The model under review builds one solid part; all positions refer to its coordinate system, in mm. Face numbers are marked on the shaded views. A direction names the side the tool comes from. Give positions to 0.01 mm unless a question says otherwise; leave off trailing zeros. Write each loop counter-clockwise with the first axis right and the second up, starting at its lowest first coordinate (ties: lowest second). Pieces come first, ordered by that corner, then holes.
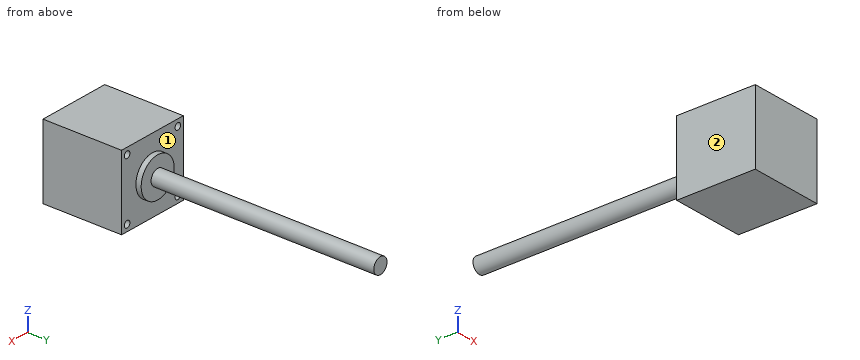
from build123d import *

# Parameters (mm, degrees)
SKETCH1_W             = 28
SKETCH1_H             = 28
BOSS_EXTRUDE1_DEPTH   = 30
SKETCH2_R             = 7.5
BOSS_EXTRUDE2_DEPTH   = 2
SKETCH3_R             = 3
BOSS_EXTRUDE3_DEPTH   = 85
SKETCH4_R             = 1
CUT_EXTRUDE1_DEPTH    = 3
M3_TAPPED_HOLE1_D     = 2.5
M3_TAPPED_HOLE1_DEPTH = 7.5
M3_TAPPED_HOLE1_TIP   = 0.751075774


with BuildPart() as part:
    # Sketch1 → Boss-Extrude1 (new body)
    with BuildSketch(Plane(origin=(0, 0, 0), x_dir=(1, 0, 0), z_dir=(0, 1, 0))):
        Rectangle(SKETCH1_W, SKETCH1_H)
    extrude(amount=BOSS_EXTRUDE1_DEPTH)

    # Sketch2 → Boss-Extrude2 (add)
    with BuildSketch(Plane(origin=(0, 30, 0), x_dir=(1, 0, 0), z_dir=(0, 1, 0))):
        with Locations(Location((0, 0, 0), (0, 0, 270))):
            Circle(SKETCH2_R)
    extrude(amount=BOSS_EXTRUDE2_DEPTH)

    # Sketch3 → Boss-Extrude3 (add)
    with BuildSketch(Plane(origin=(0, 32, 0), x_dir=(1, 0, 0), z_dir=(0, 1, 0))):
        with Locations(Location((0, 0, 0), (0, 0, 270))):
            Circle(SKETCH3_R)
    extrude(amount=BOSS_EXTRUDE3_DEPTH)

    # Sketch4 → Cut-Extrude1 (cut)
    with BuildSketch(Plane(origin=(0, 30, 0), x_dir=(1, 0, 0), z_dir=(0, 1, 0))):
        with Locations(Location((-11.5, -11.5, 0), (0, 0, 270))):
            Circle(SKETCH4_R)
        with Locations(Location((11.5, -11.5, 0), (0, 0, 270))):
            Circle(SKETCH4_R)
        with Locations(Location((-11.5, 11.5, 0), (0, 0, 270))):
            Circle(SKETCH4_R)
        with Locations(Location((11.5, 11.5, 0), (0, 0, 270))):
            Circle(SKETCH4_R)
    extrude(amount=-CUT_EXTRUDE1_DEPTH, mode=Mode.SUBTRACT)

    # M3 Tapped Hole1
    with Locations(Plane(origin=(0, 30, 0), x_dir=(1, 0, 0), z_dir=(0, 1, 0))):
        with Locations((-11.5, -11.5), (11.5, -11.5), (-11.5, 11.5), (11.5, 11.5)):
            Hole(M3_TAPPED_HOLE1_D / 2, depth=M3_TAPPED_HOLE1_DEPTH)
            with Locations((0, 0, -(M3_TAPPED_HOLE1_DEPTH + M3_TAPPED_HOLE1_TIP / 2))):  # 118° drill point
                Cone(0, M3_TAPPED_HOLE1_D / 2, M3_TAPPED_HOLE1_TIP, mode=Mode.SUBTRACT)


solid = part.part
1) Insertion check: pin 1 (1.5 mm diameter, centred on x = -11.5, z = -11.5, fed in from +Y); pin 2 (6 mm diameter, centred on y = 46, z = 1, fed in from +X); pin 3 (2 mm diameter, centred on x = 11.5, z = -11.5, fed in from +Y). Each pin has a flat end and moves straight along its axis. Give the tip position at first contact, or say it passes through.
2) Tool access review of the marked faces 1 and 2: name each direction out of +Z, -Z, +X, -X, +Y, -Y from which nothing blocks a thin tool from reaching the whole face with its end or side.
3) Consider section B-B, the plane x = -6.25. Give the boundary of the cut face in (y, z).
4) Consider section C-C, the plane y = 86. Give the boundary of the cut face in (x, z).
5) Consider section A-A, the plane z = 4.5. Give the boundary of the cut face in (x, y), then the cut area to 3 significant figures.
6) To check wall thickness, follow probe 1 along Z at (x, y) = (11.5, 26.5); probe 2 along Y at (x, z) = (-3.5, -11.5). State the ranges of each line that lie inside material, in increasing order.
7) Consider section D-D, the plane z = 0. Give the boundary of the cut face in (x, y), then the cut area to 3 significant figures.
Answer block:
1. pin 1: stops at y = 22.2
1. pin 2: stops at x = 3
1. pin 3: stops at y = 22.35
2. face 1: +Y
2. face 2: +Z, -Z, -X, +Y, -Y
3. outline: (0, -14) - (30, -14) - (30, -4.15) - (32, -4.15) - (32, 4.15) - (30, 4.15) - (30, 14) - (0, 14) - close
4. outline: circle Ø6 at (0, 0)
5. outline: (-14, 0) - (14, 0) - (14, 30) - (6, 30) - (6, 32) - (-6, 32) - (-6, 30) - (-14, 30) - close
5. area: 864 mm2
6. probe 1: z = -14 to -12.75, -10.25 to 10.25, 12.75 to 14
6. probe 2: y = 0 to 30
7. outline: (-14, 0) - (14, 0) - (14, 30) - (7.5, 30) - (7.5, 32) - (3, 32) - (3, 117) - (-3, 117) - (-3, 32) - (-7.5, 32) - (-7.5, 30) - (-14, 30) - close
7. area: 1,380 mm2
